Work out the finished part from the listing and answer in its coordinate system (mm). A direction names the side the tool comes from. Give positions to 0.01 mm unless a question says otherwise; leave off trailing zeros. Order: outer loops, then holes, each group sorted by start corner. A loop starts at its lowest first (then second) coordinate and runs counter-clockwise, first axis right, second up. Notation, with made-up numbers: M 37,79.5 L 62,79.5 A13 ccw 62,91.5 Z; hole C 40,59.5 d3. An arc over 180 degrees is marked long. One line per item, written item: value.
from build123d import *

# Parameters (mm, degrees)
EXTRUDE_1_DEPTH = 37.5


with BuildPart() as part:
    # 草图1 → 凸台-拉伸1 (new, symmetric)
    with BuildSketch(Plane.XY):
        Polygon((0, 0), (-4.5, 0), (-4.5, 6), (-1.75, 6), (-1.75, 4.4), (-2.9, 4.4), (-2.9, 1.6), (2.9, 1.6), (2.9, 4.4), (1.75, 4.4), (1.75, 6), (4.5, 6), (4.5, 0), align=None)
    extrude(amount=EXTRUDE_1_DEPTH, both=True)


solid = part.part
(1) Find the intervals of material crossed by probe 1 along X at (y, z) = (5.35, -8); probe 2 along Y at (x, z) = (-2, -7); probe 3 along X at (y, z) = (3.5, -5), in increasing order. Write a range as from..to.
Findings:
probe 1: x = -4.5..-1.75, 1.75..4.5
probe 2: y = 0..1.6, 4.4..6
probe 3: x = -4.5..-2.9, 2.9..4.5
(2) Which of the six approach directions +Z, -Z, +X, -X, +Y, -Y give full straight-line access (tool end or side, diameter ignored) to faces 1 (the flat face through (3, 6, 1)), 2 (the flat face through (-2, 4.4, 1)), 3 (the flat face through (1.75, 5, 1))?
Findings:
face 1: +Z, -Z, +X, -X, +Y
face 2: +Z, -Z
face 3: +Z, -Z, +Y
(3) Section A-A, the plane y = 3.7 is taken. Give the vertices of the cut face in (x, z), then the cut area to 3 significant figures.
Findings:
outline: M -4.5,-37.5 L -2.9,-37.5 L -2.9,37.5 L -4.5,37.5 Z; M 2.9,-37.5 L 4.5,-37.5 L 4.5,37.5 L 2.9,37.5 Z
area: 240 mm^2
(4) Section B-B, the plane z = 24 is taken. Give the vertices of the cut face in (x, y), then the cut area to 3 significant figures.
Findings:
outline: M -4.5,0 L 4.5,0 L 4.5,6 L 1.75,6 L 1.75,4.4 L 2.9,4.4 L 2.9,1.6 L -2.9,1.6 L -2.9,4.4 L -1.75,4.4 L -1.75,6 L -4.5,6 Z
area: 32.2 mm^2
(5) Section C-C, the plane x = 0.75 is taken. Give the vertices of the cut face in (y, z).
Findings:
outline: M 0,-37.5 L 1.6,-37.5 L 1.6,37.5 L 0,37.5 Z
(6) Determine the mould class of faces 4 (the flat face through (0, 1, -37.5)), 5 (the flat face through (-3, 6, 1)), 6 (the flat face through (2.9, 3, 1)), 7 (the flat face through (0, 0, 1)) for opening direction Y: pulls with the +Y half, pulls with the -Y half, needs draft (parallel to the pull), parting line crosses it, or undercut.
Findings:
face 4: needs draft
face 5: pulls with the +Y half
face 6: undercut
face 7: pulls with the -Y half
